from build123d import *

# Parameters (mm, degrees)
BOSS_EXTRUDE1_DEPTH      = 250
BOSS_EXTRUDE1_DEPTH_BACK = 250
SKETCH1_W                = 1000
SKETCH1_H                = 800
BOSS_EXTRUDE2_DEPTH      = 500
BOSS_EXTRUDE2_DEPTH_BACK = 500
SKETCH2_R                = 100
FILLET1_R                = 300
FILLET2_R                = 200


with BuildPart() as part:
    # Sketch1 → Boss-Extrude1 (new, two sides: drawn at the far end of the back side and taken through both)
    with BuildSketch(Plane.XY.offset(-BOSS_EXTRUDE1_DEPTH_BACK)):
        with Locations((200, -100)):
            Rectangle(SKETCH1_W, SKETCH1_H)
    extrude(amount=BOSS_EXTRUDE1_DEPTH + BOSS_EXTRUDE1_DEPTH_BACK)

    # Sketch2 → Boss-Extrude2 (add, two sides: drawn at the far end of the back side and taken through both)
    with BuildSketch(Plane.XY.offset(-BOSS_EXTRUDE2_DEPTH_BACK)):
        Circle(SKETCH2_R)
    extrude(amount=BOSS_EXTRUDE2_DEPTH + BOSS_EXTRUDE2_DEPTH_BACK)

    # Fillet1
    fillet1_edges = [part.edges().sort_by_distance(p)[0] for p in [
        (-300, 300, 0),
    ]]
    fillet(fillet1_edges, radius=FILLET1_R)

    # Fillet2
    fillet2_edges = [part.edges().sort_by_distance(p)[0] for p in [
        (700, 300, 0),
    ]]
    fillet(fillet2_edges, radius=FILLET2_R)


solid = part.part
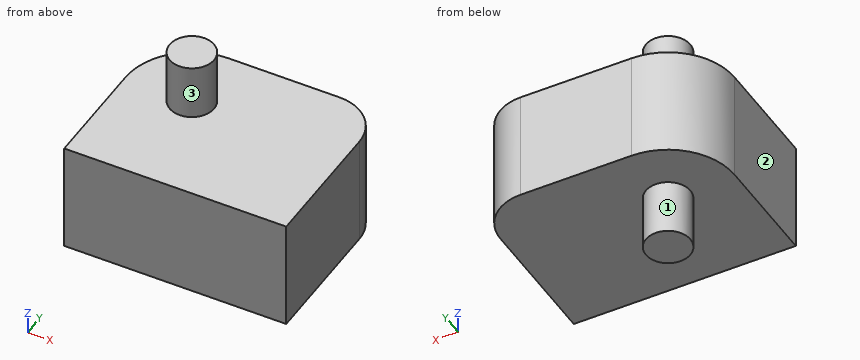
Read the model definition and answer for the solid it produces. Units are mm, in the model's axes. Face numbers are marked on the shaded views. A direction names the side the tool comes from. Give positions to 0.01 mm unless a question says otherwise; leave off trailing zeros. Loops run counter-clockwise (first coordinate to the right, second up) from the corner with the lowest first, then second, coordinate; pieces in that order, holes last. Notation, with made-up numbers: (-17, -29.5) -> (17, -29.5) arc R16 ccw to (17, -22.5) -> close; hole circle Ø10 at (13, -38.75). An arc over 180 degrees is marked (long way). Use a Markdown table: item, result.
Q1. Find the intervals of material crossed by line 1 along Z through (x, y) = (441, -455); line 2 along Y through (x, z) = (-88, -77); line 3 along Y through (x, z) = (-182, 144.5), in increasing order.
Solved:
| item | result |
|---|---|
| line 1 | z = -250 to 250 |
| line 2 | y = -500 to 286.8 |
| line 3 | y = -500 to 238.49 |
Q2. A tool of negligible diameter and unlimited length cuts with its end or side. For the marked faces 1, 2 and 3, from which of +Z, -Z, +X, -X, +Y, -Y can it reach the whole face along a straight path? Write none if from no direction.
Solved:
| item | result |
|---|---|
| face 1 | -Z |
| face 2 | +Z, -Z, -X, +Y, -Y |
| face 3 | +Z |
Q3. Section A-A, the plane x = 377.5 is taken. Determine the outline of the cut face in (y, z), then the cut area to 3 significant figures.
Solved:
| item | result |
|---|---|
| outline | (-500, -250) -> (300, -250) -> (300, 250) -> (-500, 250) -> close |
| area | 400,000 mm^2 |
Q4. Section C-C, the plane y = -287.5 is taken. Determine the outline of the cut face in (x, z).
Solved:
| item | result |
|---|---|
| outline | (-300, -250) -> (700, -250) -> (700, 250) -> (-300, 250) -> close |
Q5. Section B-B, the plane z = -65.5 is taken. Determine the outline of the cut face in (x, y), then the cut area to 3 significant figures.
Solved:
| item | result |
|---|---|
| outline | (-300, -500) -> (700, -500) -> (700, 100) arc R200 ccw to (500, 300) -> (0, 300) arc R300 ccw to (-300, 0) -> close |
| area | 772,000 mm^2 |
Q6. Each of these flat-tipped pins is pushed along its axis until it touches: pin 1 (5 mm diameter, centred on x = 260, y = -111.5, fed in from +Z); pin 2 (5 mm diameter, centred on x = 61.5, y = 175, fed in from -Z). Where does it stop, or does it pass through?
Solved:
| item | result |
|---|---|
| pin 1 | stops at z = 250 |
| pin 2 | stops at z = -250 |
Q7. Section D-D, the plane x = 56.5 is taken. Determine the outline of the cut face in (y, z).
Solved:
| item | result |
|---|---|
| outline | (-500, -250) -> (-82.51, -250) -> (-82.51, -500) -> (82.51, -500) -> (82.51, -250) -> (300, -250) -> (300, 250) -> (82.51, 250) -> (82.51, 500) -> (-82.51, 500) -> (-82.51, 250) -> (-500, 250) -> close |
